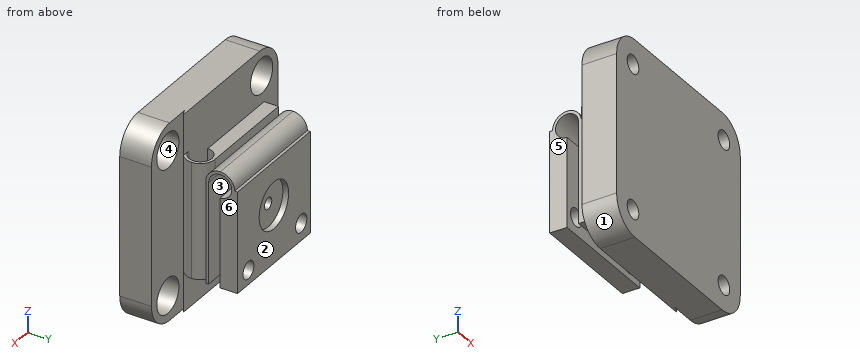
```python
from build123d import *

# Parameters (mm, degrees)
SKETCH1_W           = 34
SKETCH1_H           = 34
BOSS_EXTRUDE1_DEPTH = 6
SKETCH2_R           = 1.6
CUT_EXTRUDE1_DEPTH  = 6
SKETCH3_R           = 3.05
CUT_EXTRUDE2_DEPTH  = 4.2
SKETCH4_W           = 20
SKETCH4_H           = 20
BOSS_EXTRUDE2_DEPTH = 10
CUT_EXTRUDE4_DEPTH  = 42.243181255
CUT_EXTRUDE5_DEPTH  = 36.693136595
SKETCH7_R           = 1.5
CUT_EXTRUDE6_DEPTH  = 4
FILLET1_R           = 5
SKETCH8_R           = 1
CUT_EXTRUDE7_DEPTH  = 4
SKETCH9_R           = 4.05
CUT_EXTRUDE8_DEPTH  = 1
SKETCH10_R          = 1.55
CUT_EXTRUDE9_DEPTH  = 9


with BuildPart() as part:
    # Sketch1 → Boss-Extrude1 (new body)
    with BuildSketch(Plane(origin=(0, 0, 0), x_dir=(1, 0, 0), z_dir=(0, 1, 0))):
        Rectangle(SKETCH1_W, SKETCH1_H)
    extrude(amount=BOSS_EXTRUDE1_DEPTH)

    # Sketch2 → Cut-Extrude1 (cut)
    with BuildSketch(Plane(origin=(0, 6, 0), x_dir=(1, 0, 0), z_dir=(0, 1, 0))):
        with Locations(Location((-12.5, 12.5, 0), (0, 0, 270))):
            Circle(SKETCH2_R)
        with Locations(Location((12.5, 12.5, 0), (0, 0, 270))):
            Circle(SKETCH2_R)
        with Locations(Location((12.5, -12.5, 0), (0, 0, 270))):
            Circle(SKETCH2_R)
        with Locations(Location((-12.5, -12.5, 0), (0, 0, 270))):
            Circle(SKETCH2_R)
    extrude(amount=-CUT_EXTRUDE1_DEPTH, mode=Mode.SUBTRACT)

    # Sketch3 → Cut-Extrude2 (cut)
    with BuildSketch(Plane(origin=(0, 6, 0), x_dir=(1, 0, 0), z_dir=(0, 1, 0))):
        with Locations(Location((-12.5, 12.5, 0), (0, 0, 270))):
            Circle(SKETCH3_R)
        with Locations(Location((12.5, 12.5, 0), (0, 0, 270))):
            Circle(SKETCH3_R)
        with Locations(Location((12.5, -12.5, 0), (0, 0, 270))):
            Circle(SKETCH3_R)
        with Locations(Location((-12.5, -12.5, 0), (0, 0, 270))):
            Circle(SKETCH3_R)
    extrude(amount=-CUT_EXTRUDE2_DEPTH, mode=Mode.SUBTRACT)

    # Sketch4 → Boss-Extrude2 (add)
    with BuildSketch(Plane(origin=(0, 6, 0), x_dir=(1, 0, 0), z_dir=(0, 1, 0))):
        Rectangle(SKETCH4_W, SKETCH4_H)
    extrude(amount=BOSS_EXTRUDE2_DEPTH)

    # Sketch5 → Cut-Extrude4 (cut, through all)
    with BuildSketch(Plane.XY.offset(17)):
        with BuildLine():
            Line((-10, 6), (7.5, 6))
            ThreePointArc((7.5, 6), (8.914213562, 9.414213562), (5.5, 8))
            Line((5.5, 8), (-10, 8))
            Line((-10, 8), (-10, 6))
        make_face()
        with BuildLine():
            Line((10, 10.5), (7.5, 10.5))
            ThreePointArc((7.5, 10.5), (9.267766953, 9.767766953), (10, 8))
            Line((10, 8), (10, 10.5))
        make_face()
        with BuildLine():
            Line((10, 6), (10, 8))
            ThreePointArc((10, 8), (9.736067977, 6.881966011), (9, 6))
            Line((9, 6), (10, 6))
        make_face()
        with BuildLine():
            Line((17, 6), (10, 6))
            Line((10, 6), (9, 6))
            ThreePointArc((9, 6), (8.290569415, 5.628291755), (7.5, 5.5))
            Line((7.5, 5.5), (17, 5.5))
            Line((17, 5.5), (17, 6))
        make_face()
    extrude(amount=-CUT_EXTRUDE4_DEPTH, mode=Mode.SUBTRACT)

    # Sketch6 → Cut-Extrude5 (cut, through all)
    with BuildSketch(Plane.ZY.offset(10)):
        with BuildLine():
            ThreePointArc((10, 13), (9.267766953, 11.232233047), (7.5, 10.5))
            Line((7.5, 10.5), (10, 10.5))
            Line((10, 10.5), (10, 13))
        make_face()
        with BuildLine():
            ThreePointArc((7.5, 15.5), (9.267766953, 14.767766953), (10, 13))
            Line((10, 13), (10, 16))
            Line((10, 16), (7.5, 16))
            Line((7.5, 16), (7.5, 15.5))
        make_face()
        with BuildLine():
            Line((-10, 13), (-10, 11))
            Line((-10, 11), (7.5, 11))
            ThreePointArc((7.5, 11), (8.914213562, 14.414213562), (5.5, 13))
            Line((5.5, 13), (-10, 13))
        make_face()
    extrude(amount=-CUT_EXTRUDE5_DEPTH, mode=Mode.SUBTRACT)

    # Sketch7 → Cut-Extrude6 (cut)
    with BuildSketch(Plane(origin=(0, 16, 0), x_dir=(1, 0, 0), z_dir=(0, 1, 0))):
        with Locations(Location((7, 7.5, 0), (0, 0, 270))):
            Circle(SKETCH7_R)
    extrude(amount=-CUT_EXTRUDE6_DEPTH, mode=Mode.SUBTRACT)

    # Fillet1
    fillet1_edges = [part.edges().sort_by_distance(p)[0] for p in [
        (17, 2.75, 17),
        (17, 2.75, -17),
        (-17, 3, 17),
        (-17, 3, -17),
    ]]
    fillet(fillet1_edges, radius=FILLET1_R)

    # Sketch8 → Cut-Extrude7 (cut)
    with BuildSketch(Plane(origin=(0, 16, 0), x_dir=(1, 0, 0), z_dir=(0, 1, 0))):
        with Locations(Location((0, 0, 0), (0, 0, 270))):
            Circle(SKETCH8_R)
    extrude(amount=-CUT_EXTRUDE7_DEPTH, mode=Mode.SUBTRACT)

    # Sketch9 → Cut-Extrude8 (cut)
    with BuildSketch(Plane(origin=(0, 16, 0), x_dir=(1, 0, 0), z_dir=(0, 1, 0))):
        with Locations(Location((0, 0, 0), (0, 0, 270))):
            Circle(SKETCH9_R)
    extrude(amount=-CUT_EXTRUDE8_DEPTH, mode=Mode.SUBTRACT)

    # Sketch10 → Cut-Extrude9 (cut)
    with BuildSketch(Plane(origin=(0, 16, 0), x_dir=(1, 0, 0), z_dir=(0, 1, 0))):
        with Locations(Location((-7.5, 7, 0), (0, 0, 270))):
            Circle(SKETCH10_R)
    extrude(amount=-CUT_EXTRUDE9_DEPTH, mode=Mode.SUBTRACT)


solid = part.part
```
Build history of the part. All positions in model axes, mm. Face numbers are marked on the shaded views. A direction names the side the tool comes from. Give positions to 0.01 mm unless a question says otherwise; leave off trailing zeros. Loops run counter-clockwise (first coordinate to the right, second up) from the corner with the lowest first, then second, coordinate; pieces in that order, holes last.
1) Two-plate mould, pull along Y, no slides. Class the marked faces 1, 2 and 3: released by +Y, released by -Y, zero draft, split by the parting line, or undercut.
Values follow:
face 1: zero draft
face 2: released by +Y
face 3: undercut
2) Band-saw the part on A-A on z = 0. List the corners of the cut face in (x, y), then the cut area to 3 significant figures.
Values follow:
outline: (-17, 0) - (17, 0) - (17, 5.5) - (7.5, 5.5) arc R2.5 ccw to (7.5, 10.5) - (10, 10.5) - (10, 11) - (-10, 11) - (-10, 8) - (5.5, 8) arc R2 cw (long way) to (7.5, 6) - (-17, 6) - close; (-10, 13) - (-1, 13) - (-1, 15) - (-4.05, 15) - (-4.05, 16) - (-10, 16) - close; (1, 13) - (10, 13) - (10, 16) - (4.05, 16) - (4.05, 15) - (1, 15) - close
area: 301 mm2
3) Probe line 1 along Y through (x, z) = (-6, -5); line 2 along Y through (x, z) = (2, 0.5); line 3 along X through (y, z) = (2.65, -12.5). List the from-to ranges inside material, lowest first.
Values follow:
line 1: y = 0 to 6, 8 to 11, 13 to 16
line 2: y = 0 to 6, 8 to 11, 13 to 15
line 3: x = -16.97 to -15.55, -9.45 to 9.45, 15.55 to 16.97
4) Band-saw the part on C-C on z = -4.5. List the corners of the cut face in (x, y), then the cut area to 3 significant figures.
Values follow:
outline: (-17, 0) - (17, 0) - (17, 5.5) - (7.5, 5.5) arc R2.5 ccw to (7.5, 10.5) - (10, 10.5) - (10, 11) - (-10, 11) - (-10, 8) - (5.5, 8) arc R2 cw (long way) to (7.5, 6) - (-17, 6) - close; (-10, 13) - (10, 13) - (10, 16) - (-10, 16) - close
area: 313 mm2
5) 3-axis set-ups, long thin cutter, end or side, ignore diameter. For the marked faces 4, 5 and 6: which of +Z, -Z, +X, -X, +Y, -Y reach the whole face in a straight line?
Values follow:
face 4: +Y
face 5: +Z, -Z, -X, +Y
face 6: +Z, -Z, +X, +Y
6) Band-saw the part on B-B on y = 2.25. List the corners of the cut face in (x, z).
Values follow:
outline: (-17, -12) arc R5 ccw to (-12, -17) - (12, -17) arc R5 ccw to (17, -12) - (17, 12) arc R5 ccw to (12, 17) - (-12, 17) arc R5 ccw to (-17, 12) - close; hole circle Ø6.1 at (-12.5, -12.5); hole circle Ø6.1 at (-12.5, 12.5); hole circle Ø6.1 at (12.5, -12.5); hole circle Ø6.1 at (12.5, 12.5)
7) Band-saw the part on D-D on x = 0. List the corners of the cut face in (y, z).
Values follow:
outline: (0, -17) - (6, -17) - (6, 17) - (0, 17) - close; (8, -10) - (11, -10) - (11, 7.5) arc R2 cw (long way) to (13, 5.5) - (13, 1) - (15, 1) - (15, 4.05) - (16, 4.05) - (16, 7.5) - (15.5, 7.5) arc R2.5 ccw to (10.5, 7.5) - (10.5, 10) - (8, 10) - close; (13, -10) - (16, -10) - (16, -4.05) - (15, -4.05) - (15, -1) - (13, -1) - close
8) Drop flat-ended pins along their axis: P1, Ø2.5, axis at y = 12.5, z = 0.5, coming from the -X side; P2, Ø5, axis at x = 12.5, z = 12.5, coming from the -Y side; P3, Ø1.5, axis at x = 3.5, y = 13, coming from the +Z side; P4, Ø7, axis at x = -12.5, z = 12.5, coming from the +Y side. Give the stop position or say it passes through.
Values follow:
P1: stops at x = -10
P2: stops at y = 0
P3: stops at z = 10
P4: stops at y = 6
